The drawing under review shows one solid part. Ordinate dimensions are in mm from its lowest x, y, z. A direction names the side the tool comes from. Give positions to 0.01 mm unless a question says otherwise; leave off trailing zeros. Write each loop counter-clockwise with the first axis right and the second up, starting at its lowest first coordinate (ties: lowest second). Pieces come first, ordered by that corner, then holes. Notation, with made-up numbers: (39.25, 85.25) -> (43.25, 85.25) arc R23 ccw to (43.25, 115.25) -> close; hole circle Ø5 at (68, 4). An arc over 180 degrees is marked (long way). Answer as a JSON object with one key per item and string values.
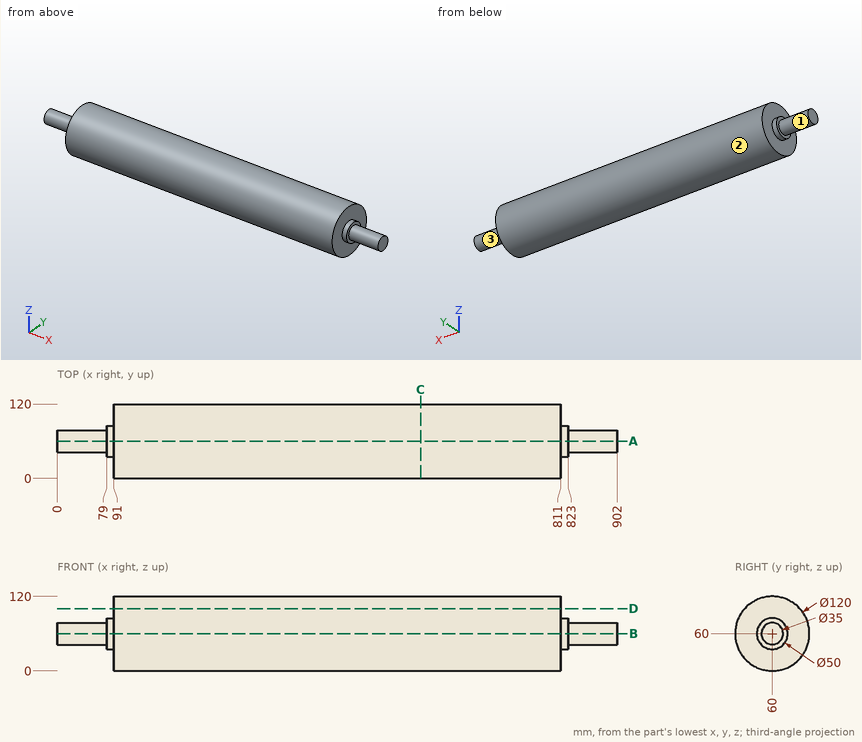
(1) We need section A-A, the plane y = 60. State the section outline as (x, z) points, then the cut area to 3 significant figures.
Here are the results:
{"outline": "(0, 42.5) -> (79, 42.5) -> (79, 35) -> (91, 35) -> (91, 0) -> (811, 0) -> (811, 35) -> (823, 35) -> (823, 42.5) -> (902, 42.5) -> (902, 77.5) -> (823, 77.5) -> (823, 85) -> (811, 85) -> (811, 120) -> (91, 120) -> (91, 85) -> (79, 85) -> (79, 77.5) -> (0, 77.5) -> close", "area": "93,100 mm²"}
(2) For line 1 along X through (y, z) = (37.5, 31); line 2 along X through (y, z) = (70, 82.5); line 3 along Y through (x, z) = (106, 87.5), list the stretches that pass through material, from the lowest coordinate up.
Here are the results:
{"line 1": "x = 91 to 811", "line 2": "x = 79 to 823", "line 3": "y = 6.67 to 113.33"}
(3) We need section D-D, the plane z = 100.5. State the section outline as (x, y) points, then the cut area to 3 significant figures.
Here are the results:
{"outline": "(91, 15.73) -> (811, 15.73) -> (811, 104.27) -> (91, 104.27) -> close", "area": "63,700 mm²"}
(4) For the marked faces 1, 2 and 3, list the 3-axis set-ups (+Z, -Z, +X, -X, +Y, -Y) from which the entire face can be reached by the end or side of a thin tool; tool diameter is ignored.
Here are the results:
{"face 1": "-X", "face 2": "+X, -X", "face 3": "+X"}
(5) We need section C-C, the plane x = 585.5. State the section outline as (y, z) points, then the cut area to 3 significant figures.
Here are the results:
{"outline": "circle Ø120 at (60, 60)", "area": "11,300 mm²"}
(6) Clearance check with flat-ended pins moving along their axes: pin 1 (1 mm diameter, centred on x = 204, y = 58, fed in from -Z); pin 2 (1.5 mm diameter, centred on x = 280.5, z = 86, fed in from -Y); pin 3 (6 mm diameter, centred on x = 125.5, z = 48.5, fed in from -Y). State where each tip first meets the part, or that it passes through.
Here are the results:
{"pin 1": "stops at z = 0.02", "pin 2": "stops at y = 5.57", "pin 3": "stops at y = 0.61"}
